Input: part model. Units: mm. Frame: model coordinates. A direction names the side the tool comes from. Round coordinates to 2 decimals unless told otherwise and drop trailing zeros. Order: outer loops, then holes, each group sorted by start corner. A loop starts at its lowest first (then second) coordinate and runs counter-clockwise, first axis right, second up.
Item 1: Cut plane A-A on z = 40. Output: boundary loops of the cut face in (x, y).
Item 2: Line query: L1, parallel to Z at x = 108, y = 24; L2, parallel to Z at x = 60, y = 15; L3, parallel to X at y = 9.25, z = 40. Output: solid intervals per line, ascending.
Item 3: Cut plane B-B on x = 60. Output: boundary loops of the cut face in (y, z), then the cut area to 3 significant figures.
Item 4: Mould query, pull axis X, two halves, no side actions, for faces 1 (the flat face through (0, 10, 15)), 2 (the flat face through (120, 10, 65)), 3 (the flat face through (61, 16, 80)), 4 (the flat face through (55, 3, 13)). Classes: released by +X, released by -X, zero draft, split by the parting line, or undercut.
Item 5: Cut plane D-D on y = 33.5. Output: boundary loops of the cut face in (x, z), then the cut area to 3 significant figures.
Item 6: First-contact query: pin 1 (13 mm diameter, centred on x = 59, z = 69.5, fed in from +Y); pin 2 (5 mm diameter, centred on y = 33, z = 54.5, fed in from -X); pin 3 (3 mm diameter, centred on y = 31, z = 13.5, fed in from -X). Flat tips, straight axial feed; report the tip coordinate or a pass-through.
Item 7: Cut plane C-C on z = 59. Output: boundary loops of the cut face in (x, y), then the cut area to 3 significant figures.
Item 8: Reachability of faces 5 (the flat face through (13, 19, 30)), 6 (the flat face through (81, 35, 39)), 7 (the flat face through (100, 5, 40)), 8 (the flat face through (65, 2, 13)) from +Z, -Z, +X, -X, +Y, -Y: full face, straight path, thin tool, end or side. Return the list, or none.
```python
from build123d import *

# Parameters (mm, degrees)
BLOCK_BODY_EXTRUDE_80_DEPTH     = 80
THROUGH_CUT_SKETCH_R            = 15
THROUGH_CUT_80_DEPTH            = 80
PROFILE_CUT_30_DEPTH            = 30
POCKET_A_SKETCH_30X30_W         = 20
POCKET_A_SKETCH_30X30_H         = 20
SQUARE_POCKET_A_30X30X20_DEPTH  = 20
POCKET_A_EXTENSION_SKETCH_W     = 28.050217784
POCKET_A_EXTENSION_SKETCH_H     = 20
POCKET_A_EXTENSION_CUT_20_DEPTH = 20
POCKET_B_SKETCH_30X30_W         = 20
POCKET_B_SKETCH_30X30_H         = 20
SQUARE_POCKET_B_30X30X20_DEPTH  = 20
POCKET_B_EXTENSION_SKETCH_W     = 28.181918945
POCKET_B_EXTENSION_SKETCH_H     = 20
POCKET_B_EXTENSION_CUT_20_DEPTH = 20


with BuildPart() as part:
    # Block Profile Sketch → Block Body Extrude 80 (new body)
    with BuildSketch(Plane.XY):
        Polygon((0, 0), (0, 20), (24, 40), (39, 40), (39, 30), (54, 30), (66, 30), (81, 30), (81, 40), (96, 40), (120, 20), (120, 0), (65, 0), (65, 5), (55, 5), (55, 0), align=None)
    extrude(amount=BLOCK_BODY_EXTRUDE_80_DEPTH)

    # Through Cut Sketch → Through Cut 80 (cut)
    with BuildSketch(Plane(origin=(0, 30, 0), x_dir=(1, 0, 0), z_dir=(0, 1, 0))):
        with Locations(Location((60, -40, 0), (0, 0, 270))):
            Circle(THROUGH_CUT_SKETCH_R)
    extrude(amount=-THROUGH_CUT_80_DEPTH, mode=Mode.SUBTRACT)

    # Profile Cut Sketch → Profile Cut 30 (cut)
    with BuildSketch(Plane.XY.offset(80)):
        Polygon((60, 30), (66, 30), (66, 22), (54, 22), (54, 30), align=None)
    extrude(amount=-PROFILE_CUT_30_DEPTH, mode=Mode.SUBTRACT)

    # Pocket A Sketch 30x30 → Square Pocket A 30x30x20 (cut)
    with BuildSketch(Plane(origin=(120, 0, 0), x_dir=(0, 0, -1), z_dir=(1, 0, 0))):
        with Locations((-40, 10)):
            Rectangle(POCKET_A_SKETCH_30X30_W, POCKET_A_SKETCH_30X30_H)
    extrude(amount=-SQUARE_POCKET_A_30X30X20_DEPTH, mode=Mode.SUBTRACT)

    # Pocket A Extension Sketch → Pocket A Extension Cut 20 (cut)
    with BuildSketch(Plane(origin=(59.016393443, 70.819672131, 0), x_dir=(0.7682212795973757, -0.6401843996644799, 0), z_dir=(0.6401843996644799, 0.7682212795973757, 0))):
        with Locations((65.357756666, -40)):
            Rectangle(POCKET_A_EXTENSION_SKETCH_W, POCKET_A_EXTENSION_SKETCH_H)
    extrude(amount=-POCKET_A_EXTENSION_CUT_20_DEPTH, mode=Mode.SUBTRACT)

    # Pocket B Sketch 30x30 → Square Pocket B 30x30x20 (cut)
    with BuildSketch(Plane.ZY):
        with Locations((40, 10)):
            Rectangle(POCKET_B_SKETCH_30X30_W, POCKET_B_SKETCH_30X30_H)
    extrude(amount=-SQUARE_POCKET_B_30X30X20_DEPTH, mode=Mode.SUBTRACT)

    # Pocket B Extension Sketch → Pocket B Extension Cut 20 (cut)
    with BuildSketch(Plane(origin=(-9.836065574, 11.803278689, 0), x_dir=(0.7682212795973757, 0.6401843996644802, 0), z_dir=(-0.64018439966448, 0.7682212795973756, 0))):
        with Locations((26.894647466, -40)):
            Rectangle(POCKET_B_EXTENSION_SKETCH_W, POCKET_B_EXTENSION_SKETCH_H)
    extrude(amount=-POCKET_B_EXTENSION_CUT_20_DEPTH, mode=Mode.SUBTRACT)


solid = part.part
```
From the geometry:
1. outline: (20, 0) - (45, 0) - (45, 30) - (39, 30) - (39, 40) - (24, 40) - (21.65, 38.04) - (34.45, 22.68) - (20, 10.63) - close; (75, 0) - (100, 0) - (100, 10.63) - (85.65, 22.59) - (98.45, 37.96) - (96, 40) - (81, 40) - (81, 30) - (75, 30) - close
2. L1: z = 0 to 30, 50 to 80
2. L2: z = 0 to 25, 55 to 80
2. L3: x = 20 to 45, 75 to 100
3. outline: (5, 0) - (30, 0) - (30, 25) - (5, 25) - close; (5, 55) - (22, 55) - (22, 80) - (5, 80) - close
3. area: 1,050 mm2
4. face 1: released by -X
4. face 2: released by +X
4. face 3: zero draft
4. face 4: undercut
5. outline: (16.2, 0) - (39, 0) - (39, 80) - (16.2, 80) - (16.2, 50) - (25.43, 50) - (25.43, 30) - (16.2, 30) - close; (81, 0) - (103.8, 0) - (103.8, 30) - (94.74, 30) - (94.74, 50) - (103.8, 50) - (103.8, 80) - (81, 80) - close
5. area: 3,280 mm2
6. pin 1: stops at y = 30
6. pin 2: stops at x = 12.6
6. pin 3: stops at x = 11.4
7. outline: (0, 0) - (55, 0) - (55, 5) - (65, 5) - (65, 0) - (120, 0) - (120, 20) - (96, 40) - (81, 40) - (81, 30) - (66, 30) - (66, 22) - (54, 22) - (54, 30) - (39, 30) - (39, 40) - (24, 40) - (0, 20) - close
7. area: 3,750 mm2
8. face 5: -X
8. face 6: +Z, -Z, +Y
8. face 7: +X, +Y, -Y
8. face 8: +Z, -Z, -Y
